Geometry: see drawing. Coordinates: mm, zero at the bounding-box minimum. A direction names the side the tool comes from. Coordinates: 2 decimals unless noted, no trailing zeros. Write each loop counter-clockwise with the first axis right and the second up, starting at its lowest first coordinate (ties: lowest second). Pieces come first, ordered by that corner, then holes. Notation, with made-up numbers: M 22.25,75.25 L 52.25,75.25 A21 cw 52.25,86.25 Z; hole C -27.5,-16 d10. An arc over 180 degrees is marked long. Answer as CSV lines item,"result". Start each with the question number.
1. Section A-A on y = 28. Return the cut outline in (x, z) (3 decimals), plus the area to 3 significant figures.
2. Reachability of the marked faces 4 and 5 from +Z, -Z, +X, -X, +Y, -Y: full face, straight path, thin tool, end or side. Return the list, or none.
3. Mould query, pull axis X, two halves, no side actions, for the marked faces 1, 2 and 3. Classes: pulls with the +X half, pulls with the -X half, needs draft (parallel to the pull), parting line crosses it, or undercut.
4. Line query: probe 1 along Y at (x, z) = (28, 5.25) (3 decimals); probe 2 along X at (y, z) = (22, 8.75); probe 3 along Y at (x, z) = (26, 10). Output: solid intervals per line, ascending. Write a range as [from, to].
5. Section C-C on z = 1.75. Return the cut outline in (x, y) (3 decimals).
6. Contact query for flat-ended pins moving along their axis: pin 1 Ø4 at (x, z) = (26, 10.5) entering from -Y; pin 2 Ø5 at (x, y) = (7.5, 50) entering from -Z; pin 3 Ø1 at (x, z) = (41.5, 2) entering from -Y. Output: stop coordinate, or through.
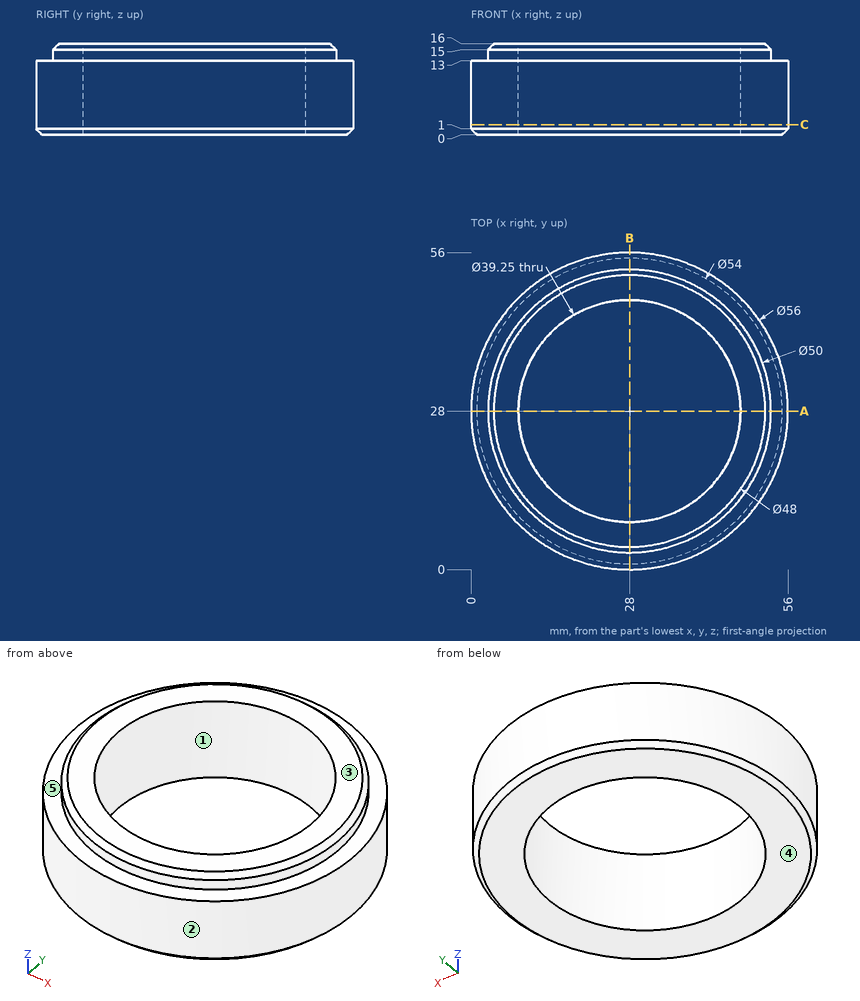
Values:
1,outline,"M 0,1 L 1,0 L 8.375,0 L 8.375,16 L 4,16 L 3,15 L 3,13 L 0,13 Z; M 47.625,0 L 55,0 L 56,1 L 56,13 L 53,13 L 53,15 L 52,16 L 47.625,16 Z"
1,area,"248 mm²"
2,face 4,"-Z, +X, -X, +Y, -Y"
2,face 5,"+Z"
3,face 1,"undercut"
3,face 2,"parting line crosses it"
3,face 3,"needs draft"
4,probe 1,"[0, 8.375], [47.625, 56]"
4,probe 2,"[0.65, 9.31], [46.69, 55.35]"
4,probe 3,"[0.07, 8.48], [47.52, 55.93]"
5,outline,"C 28,28 d56; hole C 28,28 d39.25"
6,pin 1,"y = 0"
6,pin 2,"z = 0.57"
6,pin 3,"y = 3.2"
